```python
from build123d import *

# Parameters (mm, degrees)
SKETCH_1_W                = 350
SKETCH_1_H                = 220
EXTRUDE_1_DEPTH           = 5
CUT_EXTRUDE_1_DEPTH       = 207.942020866
CUT_EXTRUDE_2_DEPTH       = 207.942020866
HOLE_WIZARD_1_D           = 6.6
HOLE_WIZARD_1_DEPTH       = 15
HOLE_WIZARD_1_CBORE_D     = 11
HOLE_WIZARD_1_CBORE_DEPTH = 6.8
HOLE_WIZARD_1_TIP         = 1.982840043
SKETCH_8_W                = 50
SKETCH_8_H                = 73
EXTRUDE_2_DEPTH           = 10
PATTERN_LINEAR_1_COUNT    = 2
PATTERN_LINEAR_1_PITCH    = 280


with BuildPart() as part:
    # 草图1 → 凸台-拉伸1 (new, symmetric)
    with BuildSketch(Plane.XY):
        Rectangle(SKETCH_1_W, SKETCH_1_H)
    extrude(amount=EXTRUDE_1_DEPTH, both=True)

    # 草图2 → 切除-拉伸1 (cut, through all)
    with BuildSketch(Plane.XY.offset(5)):
        with BuildLine():
            Line((-208, 40), (-208, -40))
            ThreePointArc((-208, -40), (-213.5, -45.5), (-219, -40))
            Line((-219, -40), (-219, 40))
            ThreePointArc((-219, 40), (-213.5, 45.5), (-208, 40))
        make_face()
        with BuildLine():
            Line((165.5, 40), (165.5, -40))
            ThreePointArc((165.5, -40), (160, -45.5), (154.5, -40))
            Line((154.5, -40), (154.5, 40))
            ThreePointArc((154.5, 40), (160, 45.5), (165.5, 40))
        make_face()
    extrude(amount=-CUT_EXTRUDE_1_DEPTH, mode=Mode.SUBTRACT)

    # 草图6 → 切除-拉伸2 (cut, through all)
    with BuildSketch(Plane.XY.offset(5)):
        with BuildLine():
            Line((98, -50), (38, -50))
            ThreePointArc((38, -50), (23.857864376, -44.142135624), (18, -30))
            Line((18, -30), (18, 30))
            ThreePointArc((18, 30), (23.857864376, 44.142135624), (38, 50))
            Line((38, 50), (98, 50))
            ThreePointArc((98, 50), (112.142135624, 44.142135624), (118, 30))
            Line((118, 30), (118, -30))
            ThreePointArc((118, -30), (112.142135624, -44.142135624), (98, -50))
        make_face()
    extrude(amount=-CUT_EXTRUDE_2_DEPTH, mode=Mode.SUBTRACT)

    # 打孔尺寸(%根据)内六角圆柱头螺钉的类型1
    with Locations(Plane(origin=(-115, 70, 5), x_dir=(1, 0, 0), z_dir=(0, 0, 1))):
        with Locations((0, 0), (0, -140), (-51, 0), (-51, -140), (-51, -70), (120, 0), (240, 0), (240, -140), (120, -140)):
            CounterBoreHole(HOLE_WIZARD_1_D / 2, HOLE_WIZARD_1_CBORE_D / 2, HOLE_WIZARD_1_CBORE_DEPTH, depth=HOLE_WIZARD_1_DEPTH)
            with Locations((0, 0, -(HOLE_WIZARD_1_DEPTH + HOLE_WIZARD_1_TIP / 2))):  # 118° drill point
                Cone(0, HOLE_WIZARD_1_D / 2, HOLE_WIZARD_1_TIP, mode=Mode.SUBTRACT)

    # 草图8 → 凸台-拉伸2 (add)
    with BuildSketch(Plane(origin=(0, 0, -5), x_dir=(-1, 0, 0), z_dir=(0, 0, -1))):
        with Locations((-150, 146.5)):
            Rectangle(SKETCH_8_W, SKETCH_8_H)
        with Locations((-150, -146.5)):
            Rectangle(SKETCH_8_W, SKETCH_8_H)
    extrude_2 = extrude(amount=-EXTRUDE_2_DEPTH)

    # 阵列(线性)1: 凸台-拉伸2 ×2
    with Locations(*[(-i * PATTERN_LINEAR_1_PITCH, 0, 0) for i in range(1, PATTERN_LINEAR_1_COUNT)]):
        add(extrude_2)


solid = part.part
```
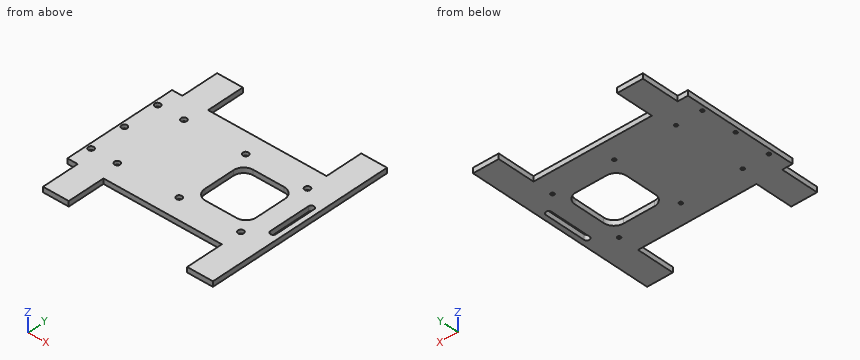
Check sheet for the modelled part. Datum: model origin and axes. Units: mm. Round coordinates to 2 decimals unless told otherwise and drop trailing zeros. Loops run counter-clockwise (first coordinate to the right, second up) from the corner with the lowest first, then second, coordinate; pieces in that order, holes last. Notation, with made-up numbers: (-27.75, 39) - (19.25, 39) arc R21 ccw to (19.25, 59) - close; hole circle Ø8 at (25, 48.25). An arc over 180 degrees is marked (long way). Answer as a JSON object with one key per item and string values. Group by question number.
Q1. Sectioned sample at C-C, the plane z = -3.5. Count the separate pieces of the cut face and the enclosed holes in it, plus the area to 3 significant figures.
Q2. Sectioned sample at D-D, the plane x = -77. Enter the section's corners in (y, z).
Q3. Gauge pin test, flat ends, axial feed: P1, Ø3.5, axis at x = -116.5, y = -71, coming from the +Z side; P2, Ø4, axis at x = -5, z = 2.5, coming from the +Y side; P3, Ø5, axis at x = 62, z = -2, coming from the -Y side. Record the tip position at first contact, or that the pin passes through.
Q4. Sectioned sample at B-B, the plane x = 43.5. Enter the section's corners in (y, z).
Q5. Scan lines: line 1 along Y through (x, z) = (-115, 3.5); line 2 along X through (y, z) = (-125.5, 3); line 3 along Y through (x, z) = (69, 0). Record each from-to range of solid material in increasing order. Write a range as [from, to].
Q6. Sectioned sample at A-A, the plane y = 142. Enter the section's corners in (x, z).
Solution:
{
 "1": {"separate pieces": "1", "enclosed holes": "11", "area": "80,700 mm²"},
 "2": {"outline": "(-110, -5) - (110, -5) - (110, 5) - (-110, 5) - close"},
 "3": {"P1": "stops at z = -1.8", "P2": "stops at y = 110", "P3": "stops at y = -110"},
 "4": {"outline": "(-110, -5) - (-50, -5) - (-50, 5) - (-110, 5) - close; (50, -5) - (110, -5) - (110, 5) - (50, 5) - close"},
 "5": {"line 1": "y = [-183, -75.5], [-64.5, 64.5], [75.5, 183]", "line 2": "x = [-155, -105], [125, 175]", "line 3": "y = [-110, -50], [50, 110]"},
 "6": {"outline": "(-155, -5) - (-105, -5) - (-105, 5) - (-155, 5) - close; (125, -5) - (175, -5) - (175, 5) - (125, 5) - close"}
}
